The listing builds one solid part. Answer for the finished solid, in the listing's coordinates (mm). A direction names the side the tool comes from. Give positions to 0.01 mm unless a question says otherwise; leave off trailing zeros. Write each loop counter-clockwise with the first axis right and the second up, starting at its lowest first coordinate (ties: lowest second). Pieces come first, ordered by that corner, then holes. Notation, with made-up numbers: M 29,39.5 L 48,39.5 A11 ccw 48,45.5 Z; hole C 20.5,-22 d9. An arc over 180 degrees is marked long. Answer as a JSON object with one key per item and string values.
```python
from build123d import *

# Parameters (mm, degrees)
BASE_PLATE_DEPTH           = 20
PIVOT_BOSS_SKETCH_R        = 35
PIVOT_BOSS_70_DEPTH        = 8
ARM_WEB_1_DEPTH            = 15
ARM_START                  = -15
ARM_WEB_2_DEPTH            = 15
LUG_START                  = 30
LUG_BOSS_1_SKETCH_R        = 26
LUG_BOSS_1_52_DEPTH        = 30
LUG_BOSS_2_SKETCH_R        = 26
LUG_BOSS_2_52_DEPTH        = 30
LUG_BORE_SKETCH_R          = 15
LUG_BORE_30_DEPTH          = 254.306139
PIVOT_COUNTERBORE_SKETCH_R = 22
PIVOT_COUNTERBORE_44_DEPTH = 13
PIVOT_HOLE_SKETCH_R        = 11
PIVOT_HOLE_22_DEPTH        = 224.494966


with BuildPart() as part:
    # Base Plate Sketch → Base Plate (new body)
    with BuildSketch(Plane(origin=(0, 0, 0), x_dir=(1, 0, 0), z_dir=(0, 1, 0))):
        with BuildLine():
            Line((0, 0), (0, 46))
            Line((0, 46), (65, 46))
            ThreePointArc((65, 46), (82.151777, 44.881636), (99.102955, 42.037041))
            Line((99.102955, 42.037041), (168.39392, 13.335784))
            ThreePointArc((168.39392, 13.335784), (190, -19), (168.39392, -51.335784))
            Line((168.39392, -51.335784), (99.102955, -80.037041))
            ThreePointArc((99.102955, -80.037041), (82.151777, -82.881636), (65, -84))
            Line((65, -84), (0, -84))
            Line((0, -84), (0, -38))
            Line((0, -38), (65, -38))
            ThreePointArc((65, -38), (84, -19), (65, 0))
            Line((65, 0), (0, 0))
        make_face()
    extrude(amount=BASE_PLATE_DEPTH)

    # Pivot Boss Sketch → Pivot Boss Ø70 (add)
    with BuildSketch(Plane(origin=(0, 20, 0), x_dir=(1, 0, 0), z_dir=(0, 1, 0))):
        with Locations(Location((155, -19, 0), (0, 0, 67.5))):
            Circle(PIVOT_BOSS_SKETCH_R)
    extrude(amount=PIVOT_BOSS_70_DEPTH)

    # Arm Web 1 Sketch → Arm Web 1 (add)
    with BuildSketch(Plane.XY.offset(84)):
        with BuildLine():
            Line((0, 0), (-44.258343, 44.258343))
            ThreePointArc((-44.258343, 44.258343), (-49.935425, 82.690681), (-11.103607, 83.858508))
            Line((-11.103607, 83.858508), (65, 20))
            Line((65, 20), (65, 0))
            Line((65, 0), (0, 0))
        make_face()
    extrude(amount=-ARM_WEB_1_DEPTH)

    # Arm Web 2 Sketch → Arm Web 2 (add)
    with BuildSketch(Plane(origin=(0, 0, -46), x_dir=(-1, 0, 0), z_dir=(0, 0, -1)).offset(ARM_START)):
        with BuildLine():
            Line((-65, 20), (-65, 0))
            Line((-65, 0), (0, 0))
            Line((0, 0), (44.258343, 44.258343))
            ThreePointArc((44.258343, 44.258343), (49.935425, 82.690681), (11.103607, 83.858508))
            Line((11.103607, 83.858508), (-65, 20))
        make_face()
    extrude(amount=ARM_WEB_2_DEPTH)

    # Lug Boss 1 Sketch → Lug Boss 1 Ø52 (add)
    with BuildSketch(Plane.XY.offset(-51).offset(LUG_START)):
        with Locations((-30, 66)):
            Circle(LUG_BOSS_1_SKETCH_R)
    extrude(amount=-LUG_BOSS_1_52_DEPTH)

    # Lug Boss 2 Sketch → Lug Boss 2 Ø52 (add)
    with BuildSketch(Plane.XY.offset(89)):
        with Locations((-30, 66)):
            Circle(LUG_BOSS_2_SKETCH_R)
    extrude(amount=-LUG_BOSS_2_52_DEPTH)

    # Lug Bore Sketch → Lug Bore Ø30 (cut, through all)
    with BuildSketch(Plane.XY.offset(89)):
        with Locations((-30, 66)):
            Circle(LUG_BORE_SKETCH_R)
    extrude(amount=-LUG_BORE_30_DEPTH, mode=Mode.SUBTRACT)

    # Pivot Counterbore Sketch → Pivot Counterbore Ø44 (cut)
    with BuildSketch(Plane(origin=(0, 28, 0), x_dir=(1, 0, 0), z_dir=(0, 1, 0))):
        with Locations(Location((155, -19, 0), (0, 0, 270))):
            Circle(PIVOT_COUNTERBORE_SKETCH_R)
    extrude(amount=-PIVOT_COUNTERBORE_44_DEPTH, mode=Mode.SUBTRACT)

    # Pivot Hole Sketch → Pivot Hole Ø22 (cut, through all)
    with BuildSketch(Plane(origin=(0, 15, 0), x_dir=(1, 0, 0), z_dir=(0, 1, 0))):
        with Locations(Location((155, -19, 0), (0, 0, 270))):
            Circle(PIVOT_HOLE_SKETCH_R)
    extrude(amount=-PIVOT_HOLE_22_DEPTH, mode=Mode.SUBTRACT)


solid = part.part
```
1. Consider line 1 along Z through (x, y) = (63, 13); line 2 along Y through (x, z) = (-30, -40.25); line 3 along Z through (x, y) = (-21, 52). Determine where each line is inside the solid, lowest interval first.
Verdict:
{"line 1": "z = -46 to 0, 38 to 84", "line 2": "y = 30 to 51, 81 to 92", "line 3": "z = -51 to -21, 59 to 89"}
2. A cutting plane is placed at A-A, the plane x = -30. Give the vertices of the cut face in (y, z), plus the area to 3 significant figures.
Verdict:
{"outline": "M 30,-46 L 40,-46 L 40,-51 L 51,-51 L 51,-21 L 40,-21 L 40,-31 L 30,-31 Z; M 30,69 L 40,69 L 40,59 L 51,59 L 51,89 L 40,89 L 40,84 L 30,84 Z; M 81,-51 L 92,-51 L 92,-21 L 81,-21 Z; M 81,59 L 92,59 L 92,89 L 81,89 Z", "area": "1,620 mm2"}
3. Flat-ended cylindrical pins translate along their axes: pin 1 (24 mm diameter, centred on x = -30, y = 66, fed in from +Z); pin 2 (4 mm diameter, centred on x = 159, z = -17.5, fed in from -Y); pin 3 (22 mm diameter, centred on x = 153.5, z = 28.5, fed in from +Y); pin 4 (5 mm diameter, centred on x = 2.5, z = -26.5, fed in from +Y). Find the tip coordinate at first contact, or state that the pin passes through.
Verdict:
{"pin 1": "passes through", "pin 2": "stops at y = 0", "pin 3": "stops at y = 15", "pin 4": "stops at y = 20"}
4. A cutting plane is placed at D-D, the plane y = 77.5. Give the vertices of the cut face in (x, z).
Verdict:
{"outline": "M -53.32,-51 L -39.63,-51 L -39.63,-21 L -53.32,-21 Z; M -53.32,59 L -39.63,59 L -39.63,89 L -53.32,89 Z; M -20.37,-51 L -6.68,-51 L -6.68,-46 L -3.53,-46 L -3.53,-31 L -6.68,-31 L -6.68,-21 L -20.37,-21 Z; M -20.37,59 L -6.68,59 L -6.68,69 L -3.53,69 L -3.53,84 L -6.68,84 L -6.68,89 L -20.37,89 Z"}
5. A cutting plane is placed at B-B, the plane y = 23. Give the vertices of the cut face in (x, z).
Verdict:
{"outline": "M -23,-46 L 61.42,-46 L 61.42,-31 L -23,-31 Z; M -23,69 L 61.42,69 L 61.42,84 L -23,84 Z; C 155,19 d70; hole C 155,19 d44"}
6. A cutting plane is placed at C-C, the plane z = 19. Give the vertices of the cut face in (x, y), plus the area to 3 significant figures.
Verdict:
{"outline": "M 84,0 L 144,0 L 144,15 L 133,15 L 133,28 L 120,28 L 120,20 L 84,20 Z; M 166,0 L 190,0 L 190,28 L 177,28 L 177,15 L 166,15 Z", "area": "1,780 mm2"}
7. The mould has two halves that part along Y. Classify faces 1 (the flat face through (-22, 22, 77)), 2 (the flat face through (23, 33, 84)), 3 (the cylindrical face through (-33.252, 51.357, 74.21)), 4 (the flat face through (150, 15, 9)): released by +Y, released by -Y, zero draft, split by the parting line, or undercut.
Verdict:
{"face 1": "released by -Y", "face 2": "zero draft", "face 3": "undercut", "face 4": "released by +Y"}
8. For faces 5 (the flat face through (0, 10, 54)), 6 (the flat face through (-19, 55, -21)), 7 (the cylindrical face through (81.91, 9.86, -44.91)), 8 (the flat face through (96, 0, 18)), 9 (the cylindrical face through (-49.163, 83.572, -35.79)), determine the directions among +Z, -Z, +X, -X, +Y, -Y from which every point of the face is accessible in a straight line to the end or side of a thin tool.
Verdict:
{"face 5": "-X, +Y, -Y", "face 6": "+X, -X, +Y, -Y", "face 7": "-Z, +X, +Y, -Y", "face 8": "+Z, -Z, +X, -X, -Y", "face 9": "none"}
